Here's how the part is built. I have some questions about the finished solid (model axes, mm). A direction names the side the tool comes from. Round coordinates to 2 decimals unless told otherwise and drop trailing zeros. Write each loop counter-clockwise with the first axis right and the second up, starting at its lowest first coordinate (ties: lowest second). Pieces come first, ordered by that corner, then holes. Notation, with made-up numbers: (-24.5, 73) -> (15.5, 73) arc R29 ccw to (15.5, 102) -> close; hole circle Ø2 at (-37, 88.5). An arc over 180 degrees is marked (long way). Answer in a Markdown table with one row per item.
from build123d import *

# Parameters (mm, degrees)
BASE_PLATE_DEPTH          = 18
UPRIGHT_PLATE_DEPTH       = 9
UPRIGHT_TOP_HOLE_SKETCH_R = 9
UPRIGHT_TOP_HOLE_18_DEPTH = 9
HUB_BOSS_SKETCH_R         = 25
HUB_BOSS_DEPTH            = 20
HUB_BORE_SKETCH_R         = 14
HUB_BORE_28_DEPTH         = 217.979261682
BASE_HOLE_SKETCH_R        = 9
BASE_HOLE_18_DEPTH        = 225.403654159
SUPPORT_RIB_REACH         = 210.435
SUPPORT_RIB_SKETCH_WALL_W = 488.071885176
SUPPORT_RIB_SKETCH_WALL_H = 10


with BuildPart() as part:
    # Base Plate Sketch → Base Plate (new body)
    with BuildSketch(Plane(origin=(0, 0, 0), x_dir=(1, 0, 0), z_dir=(0, 1, 0))):
        with BuildLine():
            Line((0, 0), (0, 53))
            ThreePointArc((0, 53), (5.272077939, 65.727922061), (18, 71))
            Line((18, 71), (78, 71))
            ThreePointArc((78, 71), (90.727922061, 65.727922061), (96, 53))
            Line((96, 53), (96, 0))
            Line((96, 0), (0, 0))
        make_face()
    extrude(amount=BASE_PLATE_DEPTH)

    # Upright Plate Sketch → Upright Plate (add)
    with BuildSketch(Plane.XY):
        with BuildLine():
            Line((0, 98), (0, 18))
            Line((0, 18), (96, 18))
            Line((96, 18), (96, 98))
            Line((96, 98), (66, 172))
            ThreePointArc((66, 172), (48, 190), (30, 172))
            Line((30, 172), (0, 98))
        make_face()
    extrude(amount=-UPRIGHT_PLATE_DEPTH)

    # Upright Top Hole Sketch → Upright Top Hole Ø18 (cut)
    with BuildSketch(Plane(origin=(0, 0, -9), x_dir=(-1, 0, 0), z_dir=(0, 0, -1))):
        with Locations((-48, 172)):
            Circle(UPRIGHT_TOP_HOLE_SKETCH_R)
    extrude(amount=-UPRIGHT_TOP_HOLE_18_DEPTH, mode=Mode.SUBTRACT)

    # Hub Boss Sketch → Hub Boss (add)
    with BuildSketch(Plane(origin=(0, 0, -9), x_dir=(-1, 0, 0), z_dir=(0, 0, -1))):
        with Locations(Location((-48, 98, 0), (0, 0, 180))):
            Circle(HUB_BOSS_SKETCH_R)
    extrude(amount=HUB_BOSS_DEPTH)

    # Hub Bore Sketch → Hub Bore Ø28 (cut, through all)
    with BuildSketch(Plane(origin=(0, 0, -29), x_dir=(-1, 0, 0), z_dir=(0, 0, -1))):
        with Locations((-48, 98)):
            Circle(HUB_BORE_SKETCH_R)
    extrude(amount=-HUB_BORE_28_DEPTH, mode=Mode.SUBTRACT)

    # Base Hole Sketch → Base Hole Ø18 (cut, through all)
    with BuildSketch(Plane.XZ):
        with Locations(Location((18, -53, 0), (0, 0, 270))):
            Circle(BASE_HOLE_SKETCH_R)
        with Locations(Location((78, -53, 0), (0, 0, 270))):
            Circle(BASE_HOLE_SKETCH_R)
    extrude(amount=-BASE_HOLE_18_DEPTH, mode=Mode.SUBTRACT)

    # Support Rib Sketch wall → Support Rib (add, up to next)
    with BuildSketch(Plane(origin=(48, 45.5, -50), x_dir=(0, -0.794767813927, -0.606913603362), z_dir=(0, 0.606913603362, -0.794767813927)), mode=Mode.PRIVATE) as support_rib_sk1:
        Rectangle(SUPPORT_RIB_SKETCH_WALL_W, SUPPORT_RIB_SKETCH_WALL_H)
    support_rib_tool1 = extrude(support_rib_sk1.sketch, amount=-SUPPORT_RIB_REACH, mode=Mode.PRIVATE) - part.part
    add(support_rib_tool1.solids().sort_by_distance((48, 45.5, -50))[0])


solid = part.part
1) I want a section at C-C, the plane z = -32. List the corners of the cut face in (x, y) for me, and give its area (3 significant figures).
Response:
| item | result |
|---|---|
| outline | (0, 0) -> (96, 0) -> (96, 18) -> (53, 18) -> (53, 69.07) -> (43, 69.07) -> (43, 18) -> (0, 18) -> close |
| area | 2,240 mm^2 |
2) I want a section at D-D, the plane y = 59. List the corners of the cut face in (x, z) for me.
Response:
| item | result |
|---|---|
| outline | (0, -9) -> (43, -9) -> (43, -39.69) -> (53, -39.69) -> (53, -9) -> (96, -9) -> (96, 0) -> (0, 0) -> close |
3) I want a section at A-A, the plane x = 59. List the corners of the cut face in (y, z) for me.
Response:
| item | result |
|---|---|
| outline | (0, -71) -> (18, -71) -> (18, -9) -> (75.55, -9) -> (75.55, -29) -> (89.34, -29) -> (89.34, 0) -> (0, 0) -> close; (106.66, -29) -> (120.45, -29) -> (120.45, -9) -> (186.25, -9) -> (186.25, 0) -> (106.66, 0) -> close |
4) We'd pull the mould along Y, two halves only. Please class faces 1 (the face through (49, 0, -36)), 2 (the face through (47, 75, 0)), 3 (the face through (48, 190, -4)), 4 (the face through (22, 18, -40)): +Y half, -Y half, draft (parallel to the pull), parting line (faces both ways), or undercut.
Response:
| item | result |
|---|---|
| face 1 | -Y half |
| face 2 | draft |
| face 3 | +Y half |
| face 4 | undercut |
5) I want a section at B-B, the plane y = 93. List the corners of the cut face in (x, z) for me.
Response:
| item | result |
|---|---|
| outline | (0, -9) -> (23.51, -9) -> (23.51, -29) -> (34.92, -29) -> (34.92, 0) -> (0, 0) -> close; (61.08, -29) -> (72.49, -29) -> (72.49, -9) -> (96, -9) -> (96, 0) -> (61.08, 0) -> close |
6) Which directions (+Z, -Z, +X, -X, +Y, -Y) give clear straight access to the entire face, cutting with the end or side of a thin tool? Please do faces 5 (the face through (43, 40, -31)), 6 (the face through (59, 109, -29)), 7 (the face through (5.133, 8.874, -65.587)), 8 (the face through (37, 67, -9)), 9 (the face through (75, 18, -40)).
Response:
| item | result |
|---|---|
| face 5 | -Z, -X |
| face 6 | -Z, +X, -X, +Y |
| face 7 | -Z, -X, +Y, -Y |
| face 8 | -Z |
| face 9 | -Z, +X |
7) I need wall thicknesses on line 1 (X direction, y = 5.25, z = -53); line 2 (Y direction, x = 48, z = -22.25); line 3 (Z direction, x = 86.5, y = 79). Which ranges of each line are inside material? Lowest first, please. Write a range as [from, to].
Response:
| item | result |
|---|---|
| line 1 | x = [0, 9], [27, 69], [87, 96] |
| line 2 | y = [0, 84], [112, 123] |
| line 3 | z = [-9, 0] |
8) For pin 1 (13 mm diameter, centred on x = 69, z = -31.5, fed in from +Y); pin 2 (14.5 mm diameter, centred on x = 78, z = -53, fed in from +Y); pin 3 (1.5 mm diameter, centred on y = 52.5, z = -10.5, fed in from +X); pin 4 (2 mm diameter, centred on x = 38, z = -8, fed in from +Y), each with a flat end and sliding along its axis, tell me the tip position at first contact or that it passes through.
Response:
| item | result |
|---|---|
| pin 1 | stops at y = 118 |
| pin 2 | passes through |
| pin 3 | stops at x = 53 |
| pin 4 | stops at y = 187.59 |
